Part model, mm, in its own coordinate system. Round coordinates to 2 decimals unless told otherwise and drop trailing zeros. Loops run counter-clockwise (first coordinate to the right, second up) from the corner with the lowest first, then second, coordinate; pieces in that order, holes last. Notation, with made-up numbers: M -17.75,18.25 L 5.25,18.25 A25 ccw 5.25,34.25 Z; hole C 3,41.5 d4. An arc over 180 degrees is marked long. Put each result on its own line as item: value. Start each with the question number.
1) Pull direction X, two halves, no side cores. Call faces 1 (the cylindrical face through (5, 0, 12)), 2 (the flat face through (-13.5, 0, 10)), 3 (the flat face through (-3, 0, 0)), 4 (the flat face through (11, 0, 17.5)): +X half, -X half, draft (parallel to the pull), parting line (faces both ways), or undercut.
2) Slice it at C-C on y = -0.7. Give the cut face in (x, z).
3) Slice it at B-B on z = 12. Give the cut face in (x, y).
4) Probe line 1 along Z through (x, y) = (6.5, 0.9); line 2 along X through (y, z) = (1.5, 10); line 3 along X through (y, z) = (-2.6, 11.5). List the from-to ranges inside material, lowest first.
5) Slice it at D-D on z = 2.75. Give the cut face in (x, y).
6) Slice it at A-A on x = 6.5. Give the cut face in (y, z), then the cut area to 3 significant figures.
```python
from build123d import *

# Parameters (mm, degrees)
SKETCH_1_W             = 27
SKETCH_1_H             = 6
EXTRUDE_1_DEPTH        = 20
HOLE_WIZARD_M6_1_D     = 5
HOLE_WIZARD_M6_1_DEPTH = 15
HOLE_WIZARD_M6_1_TIP   = 1.502151548
CHAMFER_1_SIZE         = 5


with BuildPart() as part:
    # 草图1 → 凸台-拉伸1 (new body)
    with BuildSketch(Plane.XY):
        Rectangle(SKETCH_1_W, SKETCH_1_H)
    extrude(amount=EXTRUDE_1_DEPTH)

    # M6 螺纹孔1
    with Locations(Plane(origin=(0, 3, 0), x_dir=(1, 0, 0), z_dir=(0, 1, 0))):
        with Locations((6.5, -10)):
            Hole(HOLE_WIZARD_M6_1_D / 2, depth=HOLE_WIZARD_M6_1_DEPTH)
            with Locations((0, 0, -(HOLE_WIZARD_M6_1_DEPTH + HOLE_WIZARD_M6_1_TIP / 2))):  # 118° drill point
                Cone(0, HOLE_WIZARD_M6_1_D / 2, HOLE_WIZARD_M6_1_TIP, mode=Mode.SUBTRACT)

    # 倒角1
    chamfer_1_edges = [part.edges().sort_by_distance(p)[0] for p in [
        (13.5, 0, 20),
        (13.5, 0, 0),
    ]]
    chamfer(chamfer_1_edges, length=CHAMFER_1_SIZE)


solid = part.part
```
Recorded:
1. face 1: undercut
1. face 2: -X half
1. face 3: draft
1. face 4: +X half
2. outline: M -13.5,0 L 8.5,0 L 13.5,5 L 13.5,15 L 8.5,20 L -13.5,20 Z; hole C 6.5,10 d5
3. outline: M -13.5,-3 L 5,-3 L 5,3 L -13.5,3 Z; M 8,-3 L 13.5,-3 L 13.5,3 L 8,3 Z
4. line 1: z = 0 to 7.5, 12.5 to 20
4. line 2: x = -13.5 to 4, 9 to 13.5
4. line 3: x = -13.5 to 4.5, 8.5 to 13.5
5. outline: M -13.5,-3 L 11.25,-3 L 11.25,3 L -13.5,3 Z
6. outline: M -3,0 L 3,0 L 3,7.5 L -3,7.5 Z; M -3,12.5 L 3,12.5 L 3,20 L -3,20 Z
6. area: 90.0 mm2
